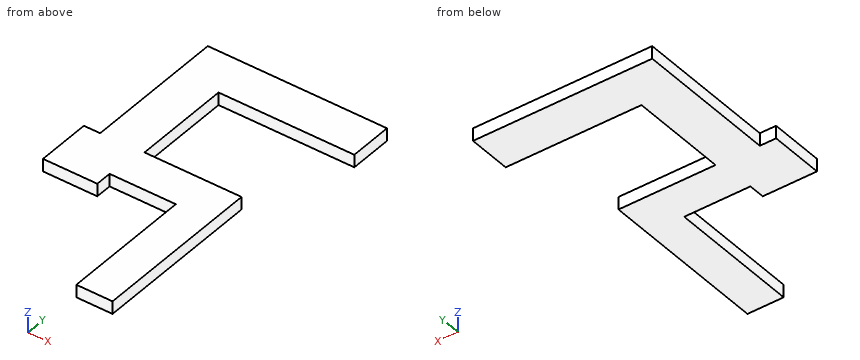
from build123d import *

# Parameters (mm, degrees)
BOSS_EXTRUDE1_DEPTH = 35


with BuildPart() as part:
    # Sketch1 → Boss-Extrude1 (new body)
    with BuildSketch(Plane.XY):
        Polygon((-495, -395), (-495, 0), (0, 0), (0, -120), (-375, -120), (-375, -391.71526804), (-107.021605816, -391.71526804), (-107.021605816, -865), (-207.021605816, -865), (-207.021605816, -500), (-390, -500), (-390, -545), (-540, -545), (-540, -395), align=None)
    extrude(amount=BOSS_EXTRUDE1_DEPTH)


solid = part.part
Part model, mm, in its own coordinate system. Round coordinates to 2 decimals unless told otherwise and drop trailing zeros. Write each loop counter-clockwise with the first axis right and the second up, starting at its lowest first coordinate (ties: lowest second). Pieces come first, ordered by that corner, then holes. Notation, with made-up numbers: (63.5, -31) - (91.5, -31) arc R11 ccw to (91.5, -12) - close; hole circle Ø10 at (40.5, 6.25). An arc over 180 degrees is marked (long way). Use CSV: the item, a comma, the result in double quotes.
Item 1: Slice it at D-D, the plane y = -261. Write the cut outline in (x, z), then the cut area to 3 significant figures.
Results list:
outline,"(-495, 0) - (-375, 0) - (-375, 35) - (-495, 35) - close"
area,"4,200 mm²"
Item 2: Slice it at C-C, the plane x = -121. Write the cut outline in (y, z).
Results list:
outline,"(-865, 0) - (-391.72, 0) - (-391.72, 35) - (-865, 35) - close; (-120, 0) - (0, 0) - (0, 35) - (-120, 35) - close"
Item 3: Slice it at B-B, the plane z = 26. Write the cut outline in (x, y).
Results list:
outline,"(-540, -545) - (-390, -545) - (-390, -500) - (-207.02, -500) - (-207.02, -865) - (-107.02, -865) - (-107.02, -391.72) - (-375, -391.72) - (-375, -120) - (0, -120) - (0, 0) - (-495, 0) - (-495, -395) - (-540, -395) - close"
Item 4: Wall check: L1, parallel to Y at x = -109.5, z = 19; L2, parallel to Y at x = -364, z = 18.5; L3, parallel to X at y = -800.5, z = 7. Give the ranges that are in metal, low to high.
Results list:
L1,"y = -865 to -391.72, -120 to 0"
L2,"y = -500 to -391.72, -120 to 0"
L3,"x = -207.02 to -107.02"
Item 5: Slice it at A-A, the plane x = -265. Write the cut outline in (y, z).
Results list:
outline,"(-500, 0) - (-391.72, 0) - (-391.72, 35) - (-500, 35) - close; (-120, 0) - (0, 0) - (0, 35) - (-120, 35) - close"
Item 6: Flat gauge pins, fed straight in: P1, Ø2, axis at x = -96, z = 14.5, coming from the -Y side; P2, Ø10.5, axis at y = -684.5, z = 12.5, coming from the +X side; P3, Ø17.5, axis at y = -226.5, z = 23, coming from the +X side; P4, Ø5, axis at x = -282.5, z = 13, coming from the +Y side. Where does each tip first touch, or does it go through?
Results list:
P1,"stops at y = -120"
P2,"stops at x = -107.02"
P3,"stops at x = -375"
P4,"stops at y = 0"
